```python
from build123d import *

# Parameters (mm, degrees)
SKETCH1_W                                           = 19
SKETCH1_H                                           = 20
SKETCH2_W                                           = 13.5
SKETCH2_H                                           = 13.5
CUT_EXTRUDE1_DEPTH                                  = 9
CBORE_FOR_M3_HEX_SOCKET_HEAD_CAP_SCREW1_D           = 3.4
CBORE_FOR_M3_HEX_SOCKET_HEAD_CAP_SCREW1_CBORE_D     = 6.5
CBORE_FOR_M3_HEX_SOCKET_HEAD_CAP_SCREW1_CBORE_DEPTH = 3.5
CUT_EXTRUDE2_DEPTH                                  = 31
SKETCH6_R                                           = 5.2
CUT_EXTRUDE3_DEPTH                                  = 3
CHAMFER1_SIZE                                       = 0.5
CHAMFER2_SIZE                                       = 1


with BuildPart() as part:
    # Sketch1 → Revolve1 (revolve)
    with BuildSketch(Plane(origin=(0, 0, 0), x_dir=(1, 0, 0), z_dir=(0, 1, 0))):
        with Locations((9.5, -10)):
            Rectangle(SKETCH1_W, SKETCH1_H)
    revolve(axis=Axis((0, 0, 0), (1, 0, 0)))

    # Sketch2 → Cut-Extrude1 (cut)
    with BuildSketch(Plane(origin=(19, 0, 0), x_dir=(0, 0, -1), z_dir=(1, 0, 0))):
        Rectangle(SKETCH2_W, SKETCH2_H)
    extrude(amount=-CUT_EXTRUDE1_DEPTH, mode=Mode.SUBTRACT)

    # CBORE for M3 Hex Socket Head Cap Screw1 (through all)
    with Locations(Plane(origin=(10, 0, 0), x_dir=(0, 0, -1), z_dir=(1, 0, 0))):
        with Locations((2.5, 0)):
            CounterBoreHole(CBORE_FOR_M3_HEX_SOCKET_HEAD_CAP_SCREW1_D / 2, CBORE_FOR_M3_HEX_SOCKET_HEAD_CAP_SCREW1_CBORE_D / 2, CBORE_FOR_M3_HEX_SOCKET_HEAD_CAP_SCREW1_CBORE_DEPTH)

    # Sketch5 → Cut-Extrude2 (cut, through all)
    with BuildSketch(Plane(origin=(10, 0, 0), x_dir=(0, 0, -1), z_dir=(1, 0, 0))):
        with BuildLine():
            Line((-2, -1), (-4, -1))
            ThreePointArc((-4, -1), (-5, 0), (-4, 1))
            Line((-4, 1), (-2, 1))
            ThreePointArc((-2, 1), (-1, 0), (-2, -1))
        make_face()
    extrude(amount=-CUT_EXTRUDE2_DEPTH, mode=Mode.SUBTRACT)

    # Sketch6 → Cut-Extrude3 (cut)
    with BuildSketch(Plane.ZY):
        Circle(SKETCH6_R)
    extrude(amount=-CUT_EXTRUDE3_DEPTH, mode=Mode.SUBTRACT)

    # Chamfer1
    chamfer1_edges = [part.edges().sort_by_distance(p)[0] for p in [
        (0, 0, -5.2),
    ]]
    chamfer(chamfer1_edges, length=CHAMFER1_SIZE)

    # Chamfer2
    chamfer2_edges = [part.edges().sort_by_distance(p)[0] for p in [
        (19, 0, 6.75),
        (19, -6.75, 0),
        (19, 0, -6.75),
        (19, 6.75, 0),
    ]]
    chamfer(chamfer2_edges, length=CHAMFER2_SIZE)


solid = part.part
```
The listing builds one solid part. Answer for the finished solid, in the listing's coordinates (mm). A direction names the side the tool comes from. Coordinates: 2 decimals unless noted, no trailing zeros. Write each loop counter-clockwise with the first axis right and the second up, starting at its lowest first coordinate (ties: lowest second). Pieces come first, ordered by that corner, then holes. Notation, with made-up numbers: (-24.5, 31.5) - (-1.5, 31.5) arc R20 ccw to (-1.5, 57.5) - close; hole circle Ø10 at (-5, 4.5). An arc over 180 degrees is marked (long way). Return JSON: item names as keys, results as strings. Group by question number.
Q1. Flat-ended cylindrical pins translate along their axes: pin 1 Ø10.5 at (y, z) = (0, -2.5) entering from -X; pin 2 Ø2.5 at (x, z) = (15, 0.5) entering from -Y; pin 3 Ø1 at (x, z) = (4.5, 9) entering from +Y; pin 4 Ø9.5 at (y, z) = (0, 0) entering from -X. Find the tip coordinate at first contact, or state that the pin passes through.
Q2. The part is cut by section B-B on x = 13.5. Write down the section's boundary in (y, z), and give its area (3 significant figures).
Q3. The part is cut by section D-D on x = 1.25. Write down the section's boundary in (y, z).
Q4. The part is cut by section A-A on y = 0. Write down the section's boundary in (x, z), and give its area (3 significant figures).
Q5. Which of the six approach directions +Z, -Z, +X, -X, +Y, -Y give full straight-line access (tool end or side, diameter ignored) to faces 5 (the cylindrical face through (1.732, 5.156, -0.677)), 6 (the flat face through (14, 6.75, 0)), 7 (the cylindrical face through (7, 0, 5))?
Q6. The part is cut by section C-C on z = 0. Write down the section's boundary in (x, y), and give its area (3 significant figures).
Q7. Find the intervals of material crossed by line 1 along Y through (x, z) = (2.25, 0); line 2 along Y through (x, z) = (15.25, 5); line 3 along Z through (x, y) = (16.75, 4.5), in increasing order. Write a range as [from, to].
Q8. For a pull along Z with two mould halves and no side action, classify faces 1 (the cylindrical face through (9.633, 19.524, -4.336)), 2 (the flat face through (14, 0, 6.75)), 3 (the flat face through (7, -1, 3)), 4 (the flat face through (0, 4.2, 4.2)) as +Z half, -Z half, draft (parallel to the pull), parting line (faces both ways), or undercut.
Evaluation:
{
 "1": {"pin 1": "stops at x = 0", "pin 2": "stops at y = -20", "pin 3": "stops at y = 18.1", "pin 4": "stops at x = 3"},
 "2": {"outline": "circle Ø40 at (0, 0); hole (-6.75, -6.75) - (6.75, -6.75) - (6.75, 6.75) - (-6.75, 6.75) - close", "area": "1,070 mm2"},
 "3": {"outline": "circle Ø40 at (0, 0); hole circle Ø10.4 at (0, 0)"},
 "4": {"outline": "(0, -20) - (19, -20) - (19, -7.75) - (18, -6.75) - (10, -6.75) - (10, -5.75) - (6.5, -5.75) - (6.5, -4.2) - (3, -4.2) - (3, -5.2) - (0.5, -5.2) - (0, -5.7) - close; (0, 5.7) - (0.5, 5.2) - (3, 5.2) - (3, 5) - (10, 5) - (10, 6.75) - (18, 6.75) - (19, 7.75) - (19, 20) - (0, 20) - close; (3, -0.8) - (6.5, -0.8) - (6.5, 0.75) - (10, 0.75) - (10, 1) - (3, 1) - close", "area": "543 mm2"},
 "5": {"face 5": "-X", "face 6": "+X", "face 7": "+X, -X"},
 "6": {"outline": "(0, -20) - (19, -20) - (19, -7.75) - (18, -6.75) - (10, -6.75) - (10, -2.08) - (6.5, -2.08) - (6.5, 2.08) - (10, 2.08) - (10, 6.75) - (18, 6.75) - (19, 7.75) - (19, 20) - (0, 20) - (0, 5.7) - (0.5, 5.2) - (3, 5.2) - (3, -5.2) - (0.5, -5.2) - (0, -5.7) - close", "area": "592 mm2"},
 "7": {"line 1": "y = [-20, -5.2], [5.2, 20]", "line 2": "y = [-19.36, -6.75], [6.75, 19.36]", "line 3": "z = [-19.49, -6.75], [6.75, 19.49]"},
 "8": {"face 1": "parting line", "face 2": "undercut", "face 3": "undercut", "face 4": "draft"}
}
